Source: CAD feature listing. Evaluate the final solid. Frame: model axes, mm. Face numbers are marked on the shaded views. A direction names the side the tool comes from. Coordinates: 2 decimals unless noted, no trailing zeros. Loops run counter-clockwise (first coordinate to the right, second up) from the corner with the lowest first, then second, coordinate; pieces in that order, holes last.
```python
from build123d import *

# Parameters (mm, degrees)
SKETCH1_W           = 60
SKETCH1_H           = 35
BOSS_EXTRUDE1_DEPTH = 10
CHAMFER1_SIZE       = 15
CHAMFER1_SIZE2      = 8.660254038
SKETCH2_W           = 36
SKETCH2_H           = 20
CUT_EXTRUDE1_DEPTH  = 37.142080737
FILLET1_R           = 2
CUT_EXTRUDE2_DEPTH  = 37.142080737
CHAMFER2_SIZE       = 1


with BuildPart() as part:
    # Sketch1 → Boss-Extrude1 (new body)
    with BuildSketch(Plane(origin=(0, 0, 0), x_dir=(1, 0, 0), z_dir=(0, 1, 0))):
        Rectangle(SKETCH1_W, SKETCH1_H)
    extrude(amount=BOSS_EXTRUDE1_DEPTH)

    # Chamfer1
    chamfer1_edges = [part.edges().sort_by_distance(p)[0] for p in [
        (0, 10, 17.5),
    ]]
    chamfer1_side = [part.faces().sort_by_distance(p)[0] for p in [
        (0, 10, 0),
    ]]
    chamfer(chamfer1_edges, length=CHAMFER1_SIZE, length2=CHAMFER1_SIZE2, reference=chamfer1_side[0])

    # Sketch2 → Cut-Extrude1 (cut, through all)
    with BuildSketch(Plane(origin=(0, 10, 0), x_dir=(1, 0, 0), z_dir=(0, 1, 0))):
        with Locations((0, -7.5)):
            Rectangle(SKETCH2_W, SKETCH2_H)
    extrude(amount=-CUT_EXTRUDE1_DEPTH, mode=Mode.SUBTRACT)

    # Fillet1
    fillet1_edges = [part.edges().sort_by_distance(p)[0] for p in [
        (-18, 5, -2.5),
        (18, 5, -2.5),
    ]]
    fillet(fillet1_edges, radius=FILLET1_R)

    # Sketch3 → Cut-Extrude2 (cut, through all)
    with BuildSketch(Plane(origin=(0, 10, 0), x_dir=(1, 0, 0), z_dir=(0, 1, 0))):
        with BuildLine():
            Line((-20.3, 13), (-20.3, 7))
            ThreePointArc((-20.3, 7), (-23, 4.3), (-25.7, 7))
            Line((-25.7, 7), (-25.7, 13))
            ThreePointArc((-25.7, 13), (-23, 15.7), (-20.3, 13))
        make_face()
    cut_extrude2 = extrude(amount=-CUT_EXTRUDE2_DEPTH, mode=Mode.SUBTRACT)

    # Mirror1: Cut-Extrude2 across plane
    add(cut_extrude2.mirror(Plane(origin=(0, 0, 0), x_dir=(0, 0, 1), z_dir=(1, 0, 0))), mode=Mode.SUBTRACT)

    # Chamfer2
    chamfer2_edges = [part.edges().sort_by_distance(p)[0] for p in [
        (-30, 5, -17.5),
        (30, 5, -17.5),
    ]]
    chamfer(chamfer2_edges, length=CHAMFER2_SIZE)


solid = part.part
```
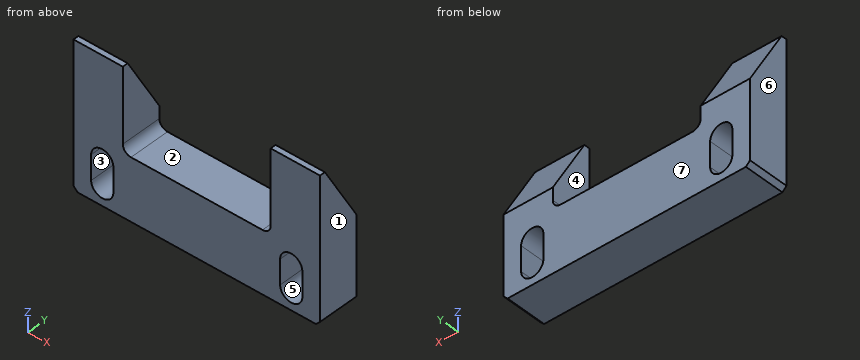
Q1. Section query C-C on y = 3.75. Return the cut outline in (x, z).
Q2. First-contact query: pin 1 Ø3 at (y, z) = (7.5, 12) entering from +X; pin 2 Ø6 at (x, z) = (16, 11.5) entering from +Y; pin 3 Ø5 at (x, y) = (21, 5) entering from +Z; pin 4 Ø2 at (y, z) = (6, 11) entering from -X. Flat tips, straight axial feed; report the tip coordinate or a pass-through.
Q3. Reachability of the marked faces 1, 2 and 3 from +Z, -Z, +X, -X, +Y, -Y: full face, straight path, thin tool, end or side. Return the list, or none.
Q4. Section query B-B on z = 5. Return the cut outline in (x, y), then the cut area to 3 significant figures.
Q5. Material intervals for line 1 along X through (y, z) = (7.25, -10); line 2 along X through (y, z) = (2.25, 8); line 3 along Z through (x, y) = (0, 2.25), sorted ascending.
Q6. Section query A-A on x = -23. Return the cut outline in (y, z).
Q7. Draft query along X for the marked faces 4, 5, 6 and 7. Return one class per face: released by +X, released by -X, zero draft, split by the parting line, or undercut.
Q8. Section query D-D on z = 14. Return the cut outline in (x, y), then the cut area to 3 significant figures.
Resolved:
1. outline: (-30, -16.5) - (-29, -17.5) - (29, -17.5) - (30, -16.5) - (30, 13.33) - (18, 13.33) - (18, -0.5) arc R2 cw to (16, -2.5) - (-16, -2.5) arc R2 cw to (-18, -0.5) - (-18, 13.33) - (-30, 13.33) - close; hole (-25.7, -13) arc R2.7 ccw to (-20.3, -13) - (-20.3, -7) arc R2.7 ccw to (-25.7, -7) - close; hole (20.3, -13) arc R2.7 ccw to (25.7, -13) - (25.7, -7) arc R2.7 ccw to (20.3, -7) - close
2. pin 1: passes through
2. pin 2: stops at y = 6.09
2. pin 3: stops at z = 15.49
2. pin 4: stops at x = -30
3. face 1: +Z, -Z, +X, +Y, -Y
3. face 2: +Z, +Y, -Y
3. face 3: +Y, -Y
4. outline: (-30, 0) - (-18, 0) - (-18, 8.56) - (-30, 8.56) - close; (18, 0) - (30, 0) - (30, 8.56) - (18, 8.56) - close
4. area: 205 mm2
5. line 1: x = -30 to -25.7, -20.3 to 20.3, 25.7 to 30
5. line 2: x = -30 to -18, 18 to 30
5. line 3: z = -17.5 to -2.5
6. outline: (0, -17.5) - (10, -17.5) - (10, -15.7) - (0, -15.7) - close; (0, -4.3) - (10, -4.3) - (10, 2.5) - (1.34, 17.5) - (0, 17.5) - close
7. face 4: undercut
7. face 5: undercut
7. face 6: released by -X
7. face 7: zero draft
8. outline: (-30, 0) - (-18, 0) - (-18, 3.36) - (-30, 3.36) - close; (18, 0) - (30, 0) - (30, 3.36) - (18, 3.36) - close
8. area: 80.7 mm2
